Study the drawing (mm; zero at the part's minimum x, y, z) and answer. A direction names the side the tool comes from. Coordinates: 2 decimals unless noted, no trailing zeros. Loops run counter-clockwise (first coordinate to the right, second up) from the corner with the lowest first, then second, coordinate; pieces in that order, holes last. Notation, with made-up numbers: (-15, 64) -> (26, 64) arc R14 cw to (26, 81) -> close; hole circle Ø1 at (-12.5, 43.5). An arc over 180 degrees is marked (long way). Answer in a Markdown table with one row per item.
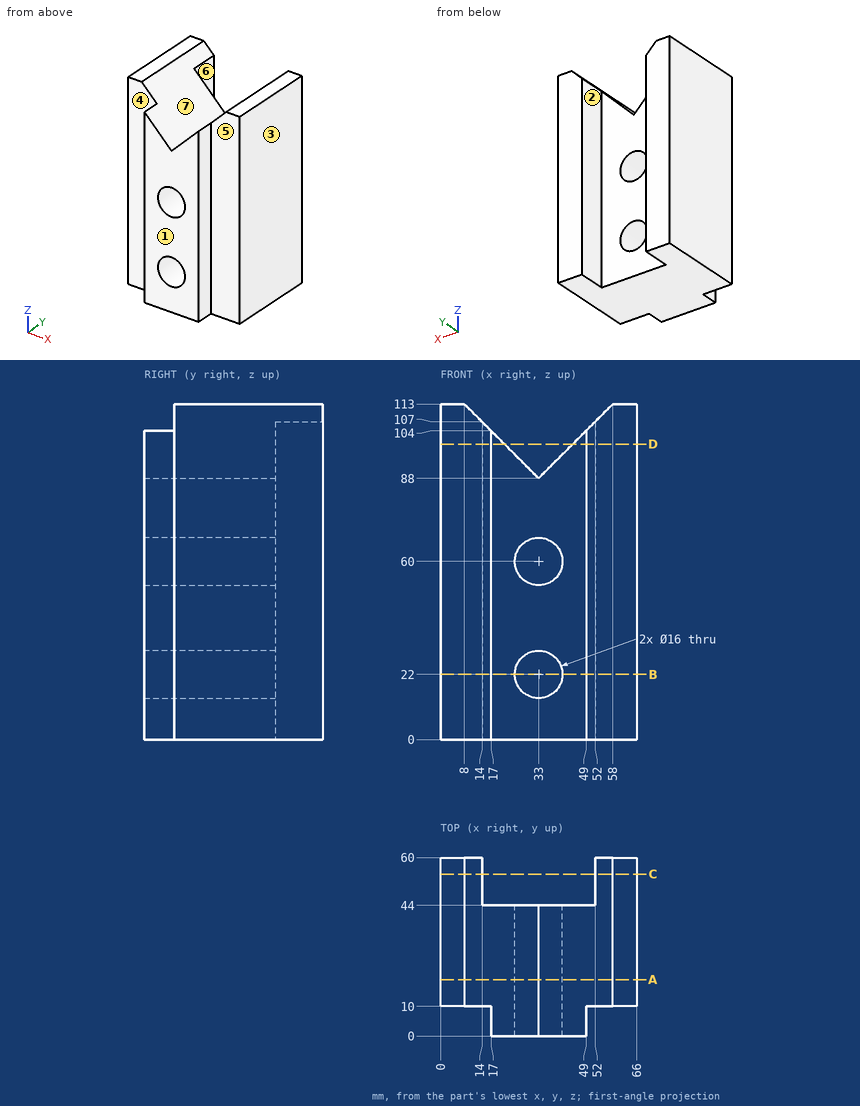
1. A cutting plane is placed at B-B on z = 22. Give the vertices of the cut face in (x, y).
A:
| item | result |
|---|---|
| outline | (0, 10) -> (17, 10) -> (17, 0) -> (25, 0) -> (25, 44) -> (14, 44) -> (14, 60) -> (0, 60) -> close; (41, 0) -> (49, 0) -> (49, 10) -> (66, 10) -> (66, 60) -> (52, 60) -> (52, 44) -> (41, 44) -> close |
2. A tool of negligible diameter and unlimited length cuts with its end or side. For the marked faces 4, 5, 6 and 7, from which of +Z, -Z, +X, -X, +Y, -Y can it reach the whole face along a straight path? Write none if from no direction.
A:
| item | result |
|---|---|
| face 4 | +Z, -Z, -X, -Y |
| face 5 | +Z, -Z, +X, -Y |
| face 6 | +Z, -Z, +Y |
| face 7 | +Z, +Y, -Y |
3. Given pin 1 Ø3 at (y, z) = (7.5, 72) entering from +X; pin 2 Ø13 at (x, z) = (33, 60) entering from +Y; pin 3 Ø2 at (x, y) = (49.5, 31) entering from +Z; pin 4 Ø18.5 at (x, z) = (59, 50.5) entering from -Y, each flat-ended and moving along its own axis, determine where each tip first touches the part or whether it passes through.
A:
| item | result |
|---|---|
| pin 1 | stops at x = 49 |
| pin 2 | passes through |
| pin 3 | stops at z = 105.5 |
| pin 4 | stops at y = 10 |
4. Find the intervals of material crossed by probe 1 along X at (y, z) = (32, 60); probe 2 along Z at (x, y) = (37.5, 12); probe 3 along Y at (x, z) = (22.5, 68.5), in increasing order.
A:
| item | result |
|---|---|
| probe 1 | x = 0 to 25, 41 to 66 |
| probe 2 | z = 0 to 15.39, 28.61 to 53.39, 66.61 to 92.5 |
| probe 3 | y = 0 to 44 |
5. A cutting plane is placed at A-A on y = 19. Give the vertices of the cut face in (x, z).
A:
| item | result |
|---|---|
| outline | (0, 0) -> (66, 0) -> (66, 113) -> (58, 113) -> (33, 88) -> (8, 113) -> (0, 113) -> close; hole circle Ø16 at (33, 22); hole circle Ø16 at (33, 60) |
6. The mould has two halves that part along X. Classify the marked faces 1, 2 and 3: pulls with the +X half, pulls with the -X half, needs draft (parallel to the pull), parting line crosses it, or undercut.
A:
| item | result |
|---|---|
| face 1 | needs draft |
| face 2 | undercut |
| face 3 | pulls with the +X half |
7. A cutting plane is placed at C-C on y = 54.5. Give the vertices of the cut face in (x, z).
A:
| item | result |
|---|---|
| outline | (0, 0) -> (14, 0) -> (14, 107) -> (8, 113) -> (0, 113) -> close; (52, 0) -> (66, 0) -> (66, 113) -> (58, 113) -> (52, 107) -> close |
8. A cutting plane is placed at D-D on z = 99.5. Give the vertices of the cut face in (x, y), and give its area (3 significant figures).
A:
| item | result |
|---|---|
| outline | (0, 10) -> (17, 10) -> (17, 0) -> (21.5, 0) -> (21.5, 44) -> (14, 44) -> (14, 60) -> (0, 60) -> close; (44.5, 0) -> (49, 0) -> (49, 10) -> (66, 10) -> (66, 60) -> (52, 60) -> (52, 44) -> (44.5, 44) -> close |
| area | 2,000 mm2 |
